```python
from build123d import *

# Parameters (mm, degrees)
HOLE_WIZARD_M3_1_D     = 2.5
HOLE_WIZARD_M3_1_DEPTH = 11.5
HOLE_WIZARD_M3_1_TIP   = 0.751075774
CHAMFER_1_SIZE         = 0.5
FILLET_1_R             = 1
SKETCH_4_W             = 0.5
SKETCH_4_H             = 23
CUT_EXTRUDE_1_DEPTH    = 5
CHAMFER_2_SIZE         = 0.2


with BuildPart() as part:
    # 草图1 → 旋转1 (revolve)
    with BuildSketch(Plane.XY, mode=Mode.PRIVATE) as revolve_1_sk:
        Polygon((1.25, 33), (1.25, 23), (4, 23), (4, 0), (0, 0), (0, 33), align=None)
    revolve(revolve_1_sk.sketch.rotate(Axis((0, -0.524377328, 0), (0, 1, 0)), 90), axis=Axis((0, -0.524377328, 0), (0, 1, 0)))

    # M3 螺纹孔1
    with Locations(Plane(origin=(0, 0, 0), x_dir=(-1, 0, 0), z_dir=(0, -1, 0))):
        with Locations((0, 0)):
            Hole(HOLE_WIZARD_M3_1_D / 2, depth=HOLE_WIZARD_M3_1_DEPTH)
            with Locations((0, 0, -(HOLE_WIZARD_M3_1_DEPTH + HOLE_WIZARD_M3_1_TIP / 2))):  # 118° drill point
                Cone(0, HOLE_WIZARD_M3_1_D / 2, HOLE_WIZARD_M3_1_TIP, mode=Mode.SUBTRACT)

    # 倒角1
    chamfer_1_edges = [part.edges().sort_by_distance(p)[0] for p in [
        (0, 0, 4),
        (0, 23, 4),
    ]]
    chamfer(chamfer_1_edges, length=CHAMFER_1_SIZE)

    # 圆角1
    fillet_1_edges = [part.edges().sort_by_distance(p)[0] for p in [
        (0, 23, 1.25),
    ]]
    fillet(fillet_1_edges, radius=FILLET_1_R)

    # 草图4 → 切除-拉伸1 (cut, symmetric)
    with BuildSketch(Plane.XY):
        with Locations((3.75, 11.5)):
            Rectangle(SKETCH_4_W, SKETCH_4_H)
        with Locations((-3.75, 11.5)):
            Rectangle(SKETCH_4_W, SKETCH_4_H)
    extrude(amount=CUT_EXTRUDE_1_DEPTH, both=True, mode=Mode.SUBTRACT)

    # 倒角2
    chamfer_2_edges = [part.edges().sort_by_distance(p)[0] for p in [
        (0, 33, 1.25),
    ]]
    chamfer(chamfer_2_edges, length=CHAMFER_2_SIZE)


solid = part.part
```
Source: CAD feature listing. Evaluate the final solid. Frame: model axes, mm. A direction names the side the tool comes from. Give positions to 0.01 mm unless a question says otherwise; leave off trailing zeros. Loops run counter-clockwise (first coordinate to the right, second up) from the corner with the lowest first, then second, coordinate; pieces in that order, holes last. Notation, with made-up numbers: (33.25, -22) -> (79.25, -22) arc R16 cw to (79.25, 8) -> close; hole circle Ø6 at (-17, 54). An arc over 180 degrees is marked (long way). Use a Markdown table: item, result. Add a question column.
(1) First-contact query: pin 1 Ø2 at (x, y) = (0, 26.5) entering from -Z; pin 2 Ø1.5 at (x, z) = (0, 0) entering from -Y. Flat tips, straight axial feed; report the tip coordinate or a pass-through.
(2) Access query for faces 4 (the face through (-0.27, 5.83, 1.22)), 5 (the face through (0.7, 23, 2.3)), 6 (the face through (0, 11, -4)). Directions: +Z, -Z, +X, -X, +Y, -Y. A direction counts if a zero-diameter tool reaches every point of the face in a straight line with its end or side. Return the directions, or none.
(3) Ray query, line 1 (Y direction, x = 2.75, z = 1.25); line 2 (Y direction, x = -1.5, z = -0.25); line 3 (X direction, y = 2, z = -1). Return the intervals inside material, ascending.
(4) Section query C-C (y = 18). Output: boundary loops of the cut face in (x, z), then the cut area to 3 significant figures.
(5) Section query B-B (y = 30). Output: boundary loops of the cut face in (x, z).
(6) Section query A-A (y = 7). Output: boundary loops of the cut face in (x, z).
(7) Pull-direction query (Z, two-part tool) for faces 1 (the face through (0, 33, 0)), 2 (the face through (-0.08, 0.135, 3.635)), 3 (the face through (0.05, 12.12, 0.21)); classes: +Z half, -Z half, draft (parallel to the pull), parting line (faces both ways), or undercut.
Checked values:
| question | item | result |
|---|---|---|
| 1 | pin 1 | z = -1.25 |
| 1 | pin 2 | y = 11.8 |
| 2 | face 4 | -Y |
| 2 | face 5 | +Y |
| 2 | face 6 | -Z, +Y, -Y |
| 3 | line 1 | 0 to 23 |
| 3 | line 2 | 0 to 23.32 |
| 3 | line 3 | -3.5 to -0.75, 0.75 to 3.5 |
| 4 | outline | (-3.5, -1.94) arc R4 ccw to (3.5, -1.94) -> (3.5, 1.94) arc R4 ccw to (-3.5, 1.94) -> close |
| 4 | area | 47.6 mm^2 |
| 5 | outline | circle Ø2.5 at (0, 0) |
| 6 | outline | (-3.5, -1.94) arc R4 ccw to (3.5, -1.94) -> (3.5, 1.94) arc R4 ccw to (-3.5, 1.94) -> close; hole circle Ø2.5 at (0, 0) |
| 7 | face 1 | draft |
| 7 | face 2 | +Z half |
| 7 | face 3 | undercut |
